from build123d import *

# Parameters (mm, degrees)
SKETCH1_R                  = 55
SKETCH1_R_2                = 30
BOSS_EXTRUDE1_DEPTH        = 34
F_17_0_17_DIAMETER_HOLE1_D = 12.6
CHAMFER1_SIZE              = 5
CHAMFER2_SIZE              = 2


with BuildPart() as part:
    # Sketch1 → Boss-Extrude1 (new body)
    with BuildSketch(Plane(origin=(0, 0, 0), x_dir=(1, 0, 0), z_dir=(0, 1, 0))):
        with Locations(Location((0, 0, 0), (0, 0, 270))):
            Circle(SKETCH1_R)
        with Locations(Location((0, 0, 0), (0, 0, 270))):
            Circle(SKETCH1_R_2, mode=Mode.SUBTRACT)
    extrude(amount=BOSS_EXTRUDE1_DEPTH)

    # Ø17.0 (17) Diameter Hole1 (through all)
    with Locations(Plane(origin=(53.62356272, 17, -12.227572173), x_dir=(0.22231949406, 0, 0.97497386763), z_dir=(0.97497386763, 0, -0.22231949406))):
        with Locations((0, 0)):
            Hole(F_17_0_17_DIAMETER_HOLE1_D / 2)

    # Chamfer1
    chamfer1_edges = [part.edges().sort_by_distance(p)[0] for p in [
        (0, 0, -55),
        (0, 34, -55),
    ]]
    chamfer(chamfer1_edges, length=CHAMFER1_SIZE)

    # Chamfer2
    chamfer2_edges = [part.edges().sort_by_distance(p)[0] for p in [
        (0, 0, -30),
        (0, 34, -30),
    ]]
    chamfer(chamfer2_edges, length=CHAMFER2_SIZE)


solid = part.part
Can you work these out from the model? Positions are in its coordinate system, mm. Coordinates: 2 decimals unless noted, no trailing zeros. Loops run counter-clockwise (first coordinate to the right, second up) from the corner with the lowest first, then second, coordinate; pieces in that order, holes last. Notation, with made-up numbers: (-19.75, 7) - (33.25, 7) arc R18 ccw to (33.25, 13) - close; hole circle Ø1 at (-24.5, -3). An arc over 180 degrees is marked (long way). Put each result on its own line as item: value. Start each with the question number.
Item 1: For pin 1 (3 mm diameter, centred on x = 26, y = 28.5, fed in from -Z); pin 2 (5 mm diameter, centred on x = -28, y = 11.5, fed in from -Z); pin 3 (6 mm diameter, centred on y = 10, z = 7, fed in from +X); pin 4 (2 mm diameter, centred on x = 34.5, z = 8.5, fed in from -Y), each with a flat end and sliding along its axis, tell me the tip position at first contact or that it passes through.
Item 2: If I drill on line 1 along X through (y, z) = (18, 0); line 2 along X through (y, z) = (28.5, 7.5); line 3 along Z through (x, y) = (-8, 2.5), over which ranges is the centre line in solid material (lowest first)?
Item 3: If we mould it in two halves opening along Y, with no side actions, what happens to faces 1 (the face through (49.815, 0.243, -6.541)), 2 (the face through (49.815, 33.757, -6.541)), 3 (the face through (41.121, 10.754, -8.535))? For each: +Y half, -Y half, draft (parallel to the pull), parting line (faces both ways), or undercut.
Item 4: Suppose I cut it at B-B (y = 12.5). Please give me the cut outline in (x, z).
Item 5: Suppose I cut it at A-A (x = 0). Please give me the cut outline in (y, z), and give its area (3 significant figures).
Item 6: Suppose I cut it at C-C (y = 26.5). Please give me the cut outline in (x, z), and give its area (3 significant figures).
Here are the results:
1. pin 1: z = -49.24
1. pin 2: z = -48.73
1. pin 3: x = 54.85
1. pin 4: y = 0
2. line 1: -55 to -30, 30 to 55
2. line 2: -54.49 to -29.05, 29.05 to 54.49
2. line 3: -51.89 to -28.91, 28.91 to 51.89
3. face 1: -Y half
3. face 2: +Y half
3. face 3: undercut
4. outline: (-54.43, 7.89) arc R55 ccw to (52.47, -16.49) - (27.95, -10.9) arc R30 cw to (-29.91, 2.3) - close; (-52.47, 16.49) - (-27.95, 10.9) arc R30 cw to (29.91, -2.3) - (54.43, -7.89) arc R55 ccw to start
5. outline: (0, -50) - (5, -55) - (29, -55) - (34, -50) - (34, -32) - (32, -30) - (2, -30) - (0, -32) - close; (0, 32) - (2, 30) - (32, 30) - (34, 32) - (34, 50) - (29, 55) - (5, 55) - (0, 50) - close
5. area: 1,640 mm²
6. outline: circle Ø110 at (0, 0); hole circle Ø60 at (0, 0)
6. area: 6,680 mm²
